The model under review builds one solid part; all positions refer to its coordinate system, in mm. Give positions to 0.01 mm unless a question says otherwise; leave off trailing zeros. Order: outer loops, then holes, each group sorted by start corner. A loop starts at its lowest first (then second) coordinate and runs counter-clockwise, first axis right, second up.
```python
from build123d import *

# Parameters (mm, degrees)
STRUCTURAL_COLD_FORMED_RECTANGULAR_HOLLO_DEPTH = 1321
SKETCH2_W                                      = 11
SKETCH2_H                                      = 22
CUT_EXTRUDE1_DEPTH                             = 676.470391653


with BuildPart() as part:
    # Sketch1 → Structural cold-formed rectangular hollow section (gb t6728-2002) 200×100×8(1) (new body)
    with BuildSketch(Plane.YZ.offset(-660.5)):
        with BuildLine():
            Line((-34, -100), (34, -100))
            ThreePointArc((34, -100), (45.313708499, -95.313708499), (50, -84))
            Line((50, -84), (50, 84))
            ThreePointArc((50, 84), (45.313708499, 95.313708499), (34, 100))
            Line((34, 100), (-34, 100))
            ThreePointArc((-34, 100), (-45.313708499, 95.313708499), (-50, 84))
            Line((-50, 84), (-50, -84))
            ThreePointArc((-50, -84), (-45.313708499, -95.313708499), (-34, -100))
        make_face()
        with BuildLine():
            Line((-34, -92), (34, -92))
            ThreePointArc((34, -92), (39.656854249, -89.656854249), (42, -84))
            Line((42, -84), (42, 84))
            ThreePointArc((42, 84), (39.656854249, 89.656854249), (34, 92))
            Line((34, 92), (-34, 92))
            ThreePointArc((-34, 92), (-39.656854249, 89.656854249), (-42, 84))
            Line((-42, 84), (-42, -84))
            ThreePointArc((-42, -84), (-39.656854249, -89.656854249), (-34, -92))
        make_face(mode=Mode.SUBTRACT)
    extrude(amount=STRUCTURAL_COLD_FORMED_RECTANGULAR_HOLLO_DEPTH)

    # Sketch2 → Cut-Extrude1 (cut, through all)
    with BuildSketch(Plane.XZ.offset(50)):
        with Locations((-655, 89)):
            Rectangle(SKETCH2_W, SKETCH2_H)
    cut_extrude1 = extrude(amount=-CUT_EXTRUDE1_DEPTH, mode=Mode.SUBTRACT)

    # Mirror1: Cut-Extrude1 across plane
    add(cut_extrude1.mirror(Plane(origin=(0, 0, 0), x_dir=(0, 0, 1), z_dir=(1, 0, 0))), mode=Mode.SUBTRACT)


solid = part.part
```
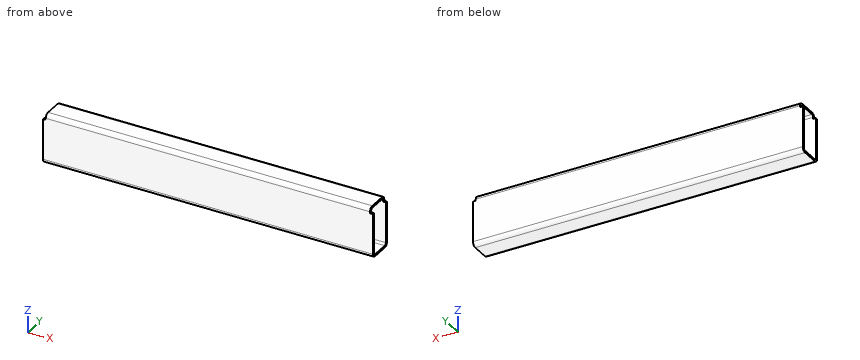
1. Take a section at B-B (z = 50). Write out the cut boundary in (x, y), and give its area (3 significant figures).
2. Take a section at A-A (y = 1). Write out the cut boundary in (x, z), and give its area (3 significant figures).
3. Take a section at C-C (x = 498). Write out the cut boundary in (y, z).
4. Insertion check: pin 1 (17.5 mm diameter, centred on y = -4.5, z = 90.5, fed in from +X); pin 2 (4 mm diameter, centred on x = -656, y = -47, fed in from +Z); pin 3 (6.5 mm diameter, centred on y = 1.5, z = 94, fed in from -X). Each pin has a flat end and moves straight along its axis. Give the tip position at first contact, or say it passes through.
5. To check wall thickness, follow line 1 (Z direction, x = 252, y = 1.5); line 2 (Y direction, x = -166.5, z = 69.5); line 3 (Z direction, x = 541, y = 41). State the ranges of each line that lie inside material, in increasing order.
Answer:
1. outline: (-660.5, -50) - (660.5, -50) - (660.5, -42) - (-660.5, -42) - close; (-660.5, 42) - (660.5, 42) - (660.5, 50) - (-660.5, 50) - close
1. area: 21,100 mm2
2. outline: (-660.5, -100) - (660.5, -100) - (660.5, -92) - (-660.5, -92) - close; (-649.5, 92) - (649.5, 92) - (649.5, 100) - (-649.5, 100) - close
2. area: 21,000 mm2
3. outline: (-50, -84) arc R16 ccw to (-34, -100) - (34, -100) arc R16 ccw to (50, -84) - (50, 84) arc R16 ccw to (34, 100) - (-34, 100) arc R16 ccw to (-50, 84) - close; hole (-42, -84) arc R8 ccw to (-34, -92) - (34, -92) arc R8 ccw to (42, -84) - (42, 84) arc R8 ccw to (34, 92) - (-34, 92) arc R8 ccw to (-42, 84) - close
4. pin 1: stops at x = 649.5
4. pin 2: stops at z = 78
4. pin 3: stops at x = -649.5
5. line 1: z = -100 to -92, 92 to 100
5. line 2: y = -50 to -42, 42 to 50
5. line 3: z = -98.39 to -87.87, 87.87 to 98.39
